from build123d import *

# Parameters (mm, degrees)
LEVER_PLATE_PROFILE_R   = 10
LEVER_PLATE_PROFILE_R_2 = 8
LEVER_PLATE_DEPTH       = 13
PIVOT_BOSS_PROFILE_R    = 8
PIVOT_BOSS_PROFILE_R_2  = 10
PIVOT_BOSSES_DEPTH      = 13.5


with BuildPart() as part:
    # Lever Plate Profile → Lever Plate (new body)
    with BuildSketch(Plane(origin=(0, 0, 0), x_dir=(1, 0, 0), z_dir=(0, 1, 0))):
        with BuildLine():
            Line((-150, -10), (0, -10))
            ThreePointArc((0, -10), (7.071067812, -7.071067812), (10, 0))
            Line((10, 0), (10, 46))
            Line((10, 46), (22, 46))
            Line((22, 46), (-7.689634159, 81.391038746))
            ThreePointArc((-7.689634159, 81.391038746), (-20.432606822, 84.806692537), (-28, 74))
            Line((-28, 74), (-28, 28))
            ThreePointArc((-28, 28), (-32.415747822, 20.255025373), (-41.329918215, 20.110018488))
            Line((-41.329918215, 20.110018488), (-110.348816191, 57.986683101))
            ThreePointArc((-110.348816191, 57.986683101), (-112.202667383, 59.389332952), (-113.574982592, 61.265750233))
            Line((-113.574982592, 61.265750233), (-135.850034815, 103.468499533))
            ThreePointArc((-135.850034815, 103.468499533), (-141.738522908, 109.702116489), (-150, 112))
            Line((-150, 112), (-150, 128))
            ThreePointArc((-150, 128), (-172.627416998, 118.627416998), (-182, 96))
            Line((-182, 96), (-178.953878866, 48.970038503))
            Line((-178.953878866, 48.970038503), (-198.20516756, 34.970038503))
            ThreePointArc((-198.20516756, 34.970038503), (-201.5, 28.5), (-198.20516756, 22.029961497))
            Line((-198.20516756, 22.029961497), (-178.953878866, 8.029961497))
            ThreePointArc((-178.953878866, 8.029961497), (-178.716545197, 7.863851996), (-178.473353106, 7.706444107))
            Line((-178.473353106, 7.706444107), (-150, -10))
        make_face()
        with Locations(Location((-150, 28.5, 0), (0, 0, 90))):
            Circle(LEVER_PLATE_PROFILE_R, mode=Mode.SUBTRACT)
        with Locations(Location((-150, 96, 0), (0, 0, 90))):
            Circle(LEVER_PLATE_PROFILE_R_2, mode=Mode.SUBTRACT)
    extrude(amount=LEVER_PLATE_DEPTH)

    # Pivot Boss Profile → Pivot Bosses (add, symmetric)
    # profile 1 of 3: a face of its own
    with BuildSketch(Plane(origin=(0, 6.5, 0), x_dir=(1, 0, 0), z_dir=(0, 1, 0))):
        with BuildLine():
            Line((-150, 112), (-150, 128))
            ThreePointArc((-150, 128), (-158.282209443, 126.909626441), (-166, 123.712812921))
            Line((-166, 123.712812921), (-166, 96))
            ThreePointArc((-166, 96), (-138.686291501, 84.686291501), (-150, 112))
        make_face()
        with Locations(Location((-150, 96, 0), (0, 0, 90))):
            Circle(PIVOT_BOSS_PROFILE_R, mode=Mode.SUBTRACT)
    # profile 2 of 3: a face of its own
    with BuildSketch(Plane(origin=(0, 6.5, 0), x_dir=(1, 0, 0), z_dir=(0, 1, 0))):
        with BuildLine():
            Line((-198.20516756, 34.970038503), (-178.953878866, 48.970038503))
            ThreePointArc((-178.953878866, 48.970038503), (-179.600430512, 36.553648048), (-167.320508076, 38.5))
            ThreePointArc((-167.320508076, 38.5), (-130, 28.5), (-167.320508076, 18.5))
            ThreePointArc((-167.320508076, 18.5), (-179.600430512, 20.446351952), (-178.953878866, 8.029961497))
            Line((-178.953878866, 8.029961497), (-198.20516756, 22.029961497))
            ThreePointArc((-198.20516756, 22.029961497), (-201.5, 28.5), (-198.20516756, 34.970038503))
        make_face()
        with Locations(Location((-150, 28.5, 0), (0, 0, 90))):
            Circle(PIVOT_BOSS_PROFILE_R_2, mode=Mode.SUBTRACT)
    # profile 3 of 3: a face of its own
    with BuildSketch(Plane(origin=(0, 6.5, 0), x_dir=(1, 0, 0), z_dir=(0, 1, 0))):
        with BuildLine():
            Line((-7.689634159, 81.391038746), (22, 46))
            Line((22, 46), (10, 46))
            Line((10, 46), (10, 38))
            Line((10, 38), (-28, 38))
            Line((-28, 38), (-28, 74))
            ThreePointArc((-28, 74), (-20.432606822, 84.806692537), (-7.689634159, 81.391038746))
        make_face()
    extrude(amount=PIVOT_BOSSES_DEPTH, both=True)


solid = part.part
Here's how the part is built. I have some questions about the finished solid (model axes, mm). A direction names the side the tool comes from. Coordinates: 2 decimals unless noted, no trailing zeros. Loops run counter-clockwise (first coordinate to the right, second up) from the corner with the lowest first, then second, coordinate; pieces in that order, holes last.
1. Imagine slicing it at D-D, the plane z = -13.5. Please give me the cut outline in (x, y), and give its area (3 significant figures).
2. For P1, Ø3.5, axis at x = -8, y = -4.5, coming from the +Z side; P2, Ø5, axis at x = -162.5, y = 0, coming from the +Z side; P3, Ø6, axis at y = 4.5, z = -97.5, coming from the -X side; P4, Ø23, axis at x = -150, z = -28.5, coming from the +Y side, each with a flat end and sliding along its axis, tell me the tip position at first contact or that it passes through.
3. I need wall thicknesses on L1, parallel to X at y = -4.5, z = -42.5; L2, parallel to X at y = 9.25, z = -28.5; L3, parallel to Y at x = -171, z = -48. Which ranges of each line are inside material? Lowest first, please.
4. If we mould it in two halves opening along X, with no side actions, what happens to faces 1 (the flat face through (-76, 6, 10)), 2 (the flat face through (6.95, 6.69, -63.94)), 3 (the flat face through (-28, 7, -51)), 4 (the flat face through (-109, 13, -28))? For each: pulls with the +X half, pulls with the -X half, needs draft (parallel to the pull), parting line crosses it, or undercut.
5. Imagine slicing it at A-A, the plane y = 17.75. Please give me the cut outline in (x, z).
6. For faces 5 (the cylindrical face through (-179.75, -3.55, -36.69)), 6 (the flat face through (10, 7, -28)), 7 (the cylindrical face through (-130.013, 16.451, -29.233)), which set-ups out of +Z, -Z, +X, -X, +Y, -Y let a thin tool reach every point of the face, with its end or its side?
7. Imagine slicing it at B-B, the plane x = -152.5. Please give me the cut outline in (y, z), and give its area (3 significant figures).
8. Imagine slicing it at C-C, the plane z = -42.5. Please give me the cut outline in (x, y).
Taken from the geometry:
1. outline: (-186.48, -7) - (-182.19, -7) - (-182.19, 0) - (-163.23, 0) - (-163.23, -7) - (-136.77, -7) - (-136.77, 0) - (10, 0) - (10, 13) - (-136.77, 13) - (-136.77, 20) - (-163.23, 20) - (-163.23, 13) - (-182.19, 13) - (-182.19, 20) - (-186.48, 20) - close
1. area: 2,980 mm2
2. P1: stops at z = -38
2. P2: stops at z = 3.78
2. P3: stops at x = -182
2. P4: stops at y = 20
3. L1: x = -187.85 to -182.25, -164.28 to -135.72, -28 to 10
3. L2: x = -201.5 to -160, -140 to -56.62, -28 to 10
3. L3: y = 0 to 13
4. face 1: needs draft
4. face 2: pulls with the +X half
4. face 3: undercut
4. face 4: undercut
5. outline: (-198.21, -34.97) - (-178.95, -48.97) arc R8 cw (long way) to (-167.32, -38.5) arc R20 ccw (long way) to (-167.32, -18.5) arc R8 cw (long way) to (-178.95, -8.03) - (-198.21, -22.03) arc R8 ccw to start; (-166, -123.71) arc R32 ccw to (-150, -128) - (-150, -112) arc R16 ccw (long way) to (-166, -96) - close; (-28, -74) arc R11.5 ccw to (-7.69, -81.39) - (22, -46) - (10, -46) - (10, -38) - (-28, -38) - close; hole circle Ø20 at (-150, -28.5); hole circle Ø16 at (-150, -96)
6. face 5: -Y
6. face 6: +Z, +X, +Y, -Y
6. face 7: +Y
7. outline: (-7, -127.9) - (20, -127.9) - (20, -103.6) - (-7, -103.6) - close; (-7, -88.4) - (20, -88.4) - (20, -80.2) - (13, -80.2) - (13, -48.34) - (20, -48.34) - (20, -38.18) - (-7, -38.18) - (-7, -48.34) - (0, -48.34) - (0, -80.2) - (-7, -80.2) - close; (-7, -18.82) - (20, -18.82) - (20, -8.66) - (13, -8.66) - (13, 8.45) - (0, 8.45) - (0, -8.66) - (-7, -8.66) - close
7. area: 2,060 mm2
8. outline: (-187.85, -7) - (-182.25, -7) - (-182.25, 0) - (-164.28, 0) - (-164.28, -7) - (-135.72, -7) - (-135.72, 0) - (-82.13, 0) - (-82.13, 13) - (-135.72, 13) - (-135.72, 20) - (-164.28, 20) - (-164.28, 13) - (-182.25, 13) - (-182.25, 20) - (-187.85, 20) - close; (-28, -7) - (10, -7) - (10, 20) - (-28, 20) - close
